Work out the finished part from the listing and answer in its coordinate system (mm). A direction names the side the tool comes from. Coordinates: 2 decimals unless noted, no trailing zeros. Loops run counter-clockwise (first coordinate to the right, second up) from the corner with the lowest first, then second, coordinate; pieces in that order, holes last. Notation, with made-up numbers: (39.25, 37.25) -> (49.25, 37.25) arc R28 cw to (49.25, 66.25) -> close; hole circle Ø11 at (-5.5, 27). An arc over 180 degrees is marked (long way). Use a Markdown table: item, result. Add a question column.
```python
from build123d import *

# Parameters (mm, degrees)
SKETCH_1_W          = 80
SKETCH_1_H          = 80
EXTRUDE_1_DEPTH     = 241
SKETCH_2_W          = 120
SKETCH_2_H          = 53
EXTRUDE_2_DEPTH     = 3
SKETCH_3_R          = 4
CUT_EXTRUDE_1_DEPTH = 262.858740545
SKETCH_4_R          = 10
CUT_EXTRUDE_2_DEPTH = 262.858740545
SKETCH_5_OUTSIDE_W  = 178.346
SKETCH_5_OUTSIDE_H  = 141.346
SKETCH_5_OUTSIDE_R  = 40
CUT_EXTRUDE_3_DEPTH = 90


with BuildPart() as part:
    # 草图1 → 凸台-拉伸1 (new body)
    with BuildSketch(Plane.XY):
        Rectangle(SKETCH_1_W, SKETCH_1_H)
    extrude(amount=EXTRUDE_1_DEPTH)

    # 草图2 → 凸台-拉伸2 (add)
    with BuildSketch(Plane(origin=(0, 40, 0), x_dir=(1, 0, 0), z_dir=(0, 1, 0))):
        with Locations((0, -26.5)):
            Rectangle(SKETCH_2_W, SKETCH_2_H)
    extrude(amount=EXTRUDE_2_DEPTH)

    # 草图3 → 切除-拉伸1 (cut, through all)
    with BuildSketch(Plane(origin=(0, 43, 0), x_dir=(1, 0, 0), z_dir=(0, 1, 0))):
        with Locations(Location((-50, -11.5, 0), (0, 0, 180))):
            Circle(SKETCH_3_R)
        with Locations(Location((50, -11.5, 0), (0, 0, 180))):
            Circle(SKETCH_3_R)
        with Locations(Location((50, -41.5, 0), (0, 0, 180))):
            Circle(SKETCH_3_R)
        with Locations(Location((-50, -41.5, 0), (0, 0, 180))):
            Circle(SKETCH_3_R)
    extrude(amount=-CUT_EXTRUDE_1_DEPTH, mode=Mode.SUBTRACT)

    # 草图4 → 切除-拉伸2 (cut, through all)
    with BuildSketch(Plane(origin=(0, 43, 0), x_dir=(1, 0, 0), z_dir=(0, 1, 0))):
        with Locations(Location((0, -26.5, 0), (0, 0, 180))):
            Circle(SKETCH_4_R)
    extrude(amount=-CUT_EXTRUDE_2_DEPTH, mode=Mode.SUBTRACT)

    # 草图5 outside → 切除-拉伸3 (cut)
    with BuildSketch(Plane.XY.offset(241)):
        with Locations((0, 1.5)):
            Rectangle(SKETCH_5_OUTSIDE_W, SKETCH_5_OUTSIDE_H)
        with Locations(Location((0, 0, 0), (0, 0, 180))):
            Circle(SKETCH_5_OUTSIDE_R, mode=Mode.SUBTRACT)
    extrude(amount=-CUT_EXTRUDE_3_DEPTH, mode=Mode.SUBTRACT)


solid = part.part
```
Item 1: Section D-D (x = -26) is taken. Determine the outline of the cut face in (y, z).
Item 2: For faces 1 (the face through (-32, 30, 151)), 2 (the face through (-50, 40, 26)), 3 (the face through (-32, -30, 151)), determine the directions among +Z, -Z, +X, -X, +Y, -Y from which every point of the face is accessible in a straight line to the end or side of a thin tool.
Item 3: Given pin 1 (7 mm diameter, centred on x = 50, z = 11.5, fed in from +Y); pin 2 (10 mm diameter, centred on x = 45.5, z = 30.5, fed in from -Y); pin 3 (10 mm diameter, centred on y = 33, z = 201, fed in from -X); pin 4 (24 mm diameter, centred on y = -3, z = 105.5, fed in from +X), each flat-ended and moving along its own axis, determine where each tip first touches the part or whether it passes through.
Item 4: Section C-C (y = -14) is taken. Determine the outline of the cut face in (x, z).
Item 5: For a pull along X with two mould halves and no side action, classify faces 4 (the face through (53.996, 41.521, 41.676)), 5 (the face through (50, 40, 26)), 6 (the face through (-40, -1, 74)) as +X half, -X half, draft (parallel to the pull), parting line (faces both ways), or undercut.
Item 6: Section B-B (x = -50) is taken. Determine the outline of the cut face in (y, z), then the cut area to 3 significant figures.
Item 7: Section A-A (z = 41.5) is taken. Determine the outline of the cut face in (x, y), then the cut area to 3 significant figures.
Item 8: Find the intervals of material crossed by probe 1 along X at (y, z) = (41, 11); probe 2 along Z at (x, y) = (50, 42.15); probe 3 along Y at (x, z) = (-15.5, 148), in increasing order.
Output:
| question | item | result |
|---|---|---|
| 1 | outline | (-40, 0) -> (43, 0) -> (43, 53) -> (40, 53) -> (40, 151) -> (30.4, 151) -> (30.4, 241) -> (-30.4, 241) -> (-30.4, 151) -> (-40, 151) -> close |
| 2 | face 1 | +Z, -X, +Y |
| 2 | face 2 | +Z, -Z, -X, -Y |
| 2 | face 3 | +Z, -X, -Y |
| 3 | pin 1 | passes through |
| 3 | pin 2 | stops at y = 40 |
| 3 | pin 3 | stops at x = -28.57 |
| 3 | pin 4 | stops at x = 40 |
| 4 | outline | (-40, 0) -> (40, 0) -> (40, 151) -> (37.47, 151) -> (37.47, 241) -> (-37.47, 241) -> (-37.47, 151) -> (-40, 151) -> close; hole circle Ø20 at (0, 26.5) |
| 5 | face 4 | undercut |
| 5 | face 5 | draft |
| 5 | face 6 | -X half |
| 6 | outline | (40, 0) -> (43, 0) -> (43, 7.5) -> (40, 7.5) -> close; (40, 15.5) -> (43, 15.5) -> (43, 37.5) -> (40, 37.5) -> close; (40, 45.5) -> (43, 45.5) -> (43, 53) -> (40, 53) -> close |
| 6 | area | 111 mm2 |
| 7 | outline | (-60, 40) -> (-54, 40) -> (-54, 43) -> (-60, 43) -> close; (-46, 40) -> (-40, 40) -> (-40, -40) -> (40, -40) -> (40, 40) -> (46, 40) -> (46, 43) -> (-46, 43) -> close; (54, 40) -> (60, 40) -> (60, 43) -> (54, 43) -> close |
| 7 | area | 6,710 mm2 |
| 8 | probe 1 | x = -60 to -53.97, -46.03 to 46.03, 53.97 to 60 |
| 8 | probe 2 | z = 0 to 7.5, 15.5 to 37.5, 45.5 to 53 |
| 8 | probe 3 | y = -40 to 40 |
